The drawing under review shows one solid part. Ordinate dimensions are in mm from its lowest x, y, z. Coordinates: 2 decimals unless noted, no trailing zeros. Order: outer loops, then holes, each group sorted by start corner. A loop starts at its lowest first (then second) coordinate and runs counter-clockwise, first axis right, second up. Notation, with made-up numbers: (76, 84) -> (121, 84) arc R13 ccw to (121, 88) -> close; hole circle Ø5 at (24, 71). An arc over 180 degrees is marked (long way). Use a Markdown table: item, result. Add a question column.
Q1. Insertion check: pin 1 (6 mm diameter, centred on x = 16.5, y = 24, fed in from -Z); pin 2 (3 mm diameter, centred on x = 23, z = 18.5, fed in from +Y). Each pin has a flat end and moves straight along its axis. Give the tip position at first contact, or say it passes through.
Q2. Wall thickness on probe 1 along Z at (x, y) = (3, 21); probe 2 along Y at (x, z) = (12, 8); probe 3 along Y at (x, z) = (7.5, 35): over which ranges is each line inside the solid? List them lowest first.
Q3. Add section C-C (z = 14.5). State the section outline as (x, y) points.
Q4. Add section A-A (x = 14.5). State the section outline as (y, z) points.
Q5. The part is to be moulded in two halves that separate along Y. For the marked faces 1, 2 and 3, say which applies: pulls with the +Y half, pulls with the -Y half, needs draft (parallel to the pull), parting line crosses it, or undercut.
Q6. Add section B-B (y = 5). State the section outline as (x, z) points.
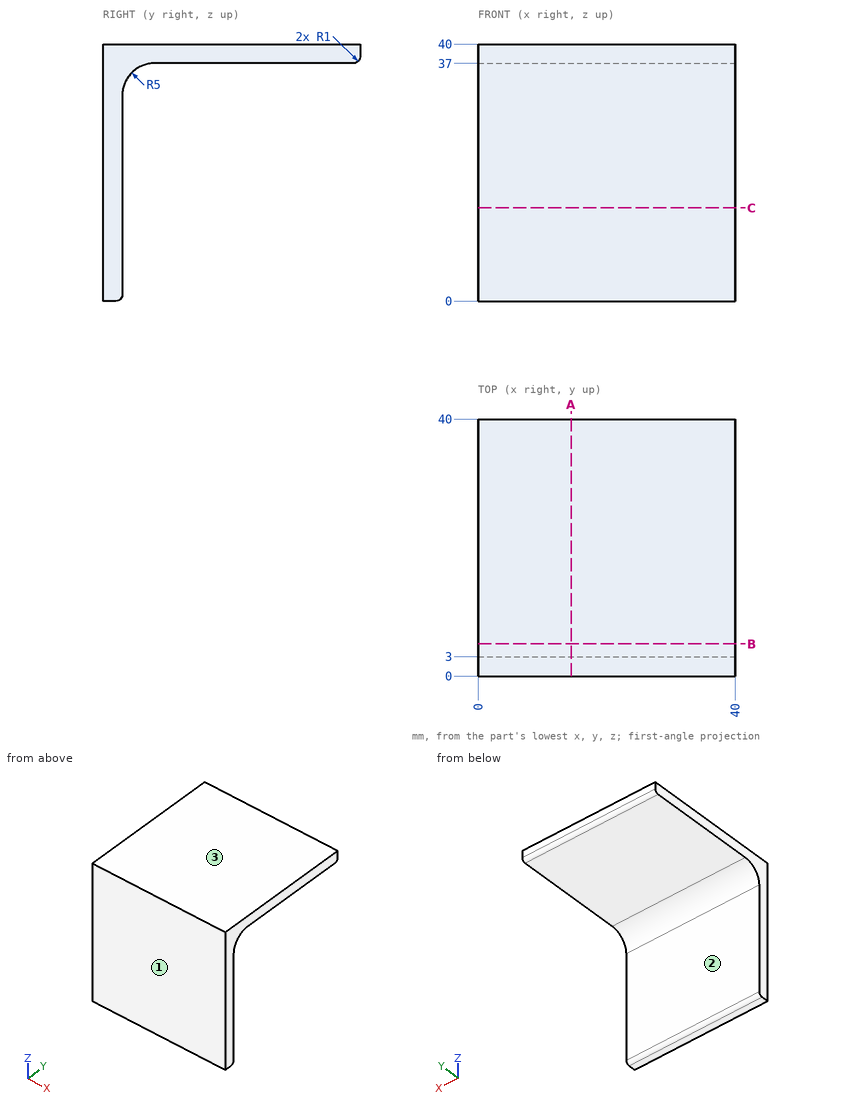
Established:
| question | item | result |
|---|---|---|
| 1 | pin 1 | z = 37 |
| 1 | pin 2 | y = 3 |
| 2 | probe 1 | 37 to 40 |
| 2 | probe 2 | 0 to 3 |
| 2 | probe 3 | 0 to 4 |
| 3 | outline | (0, 0) -> (40, 0) -> (40, 3) -> (0, 3) -> close |
| 4 | outline | (0, 0) -> (2, 0) arc R1 ccw to (3, 1) -> (3, 32) arc R5 cw to (8, 37) -> (39, 37) arc R1 ccw to (40, 38) -> (40, 40) -> (0, 40) -> close |
| 5 | face 1 | pulls with the -Y half |
| 5 | face 2 | pulls with the +Y half |
| 5 | face 3 | needs draft |
| 6 | outline | (0, 36) -> (40, 36) -> (40, 40) -> (0, 40) -> close |
